```python
from build123d import *

# Parameters (mm, degrees)
CUT_EXTRUDE1_DEPTH      = 124.693168769
CUT_EXTRUDE1_DEPTH_BACK = 124.693168769
CUT_EXTRUDE2_DEPTH      = 124.693168769


with BuildPart() as part:
    # Sketch1 → Revolve2 (revolve)
    with BuildSketch(Plane(origin=(0, 0, 0), x_dir=(0, 0, -1), z_dir=(1, 0, 0))):
        Polygon((-50, 64), (-50, 80), (0, 80), (0, 0), (-30, 0), (-30, 64), align=None)
    revolve(axis=Axis((0, 0, -85.976986238), (0, 0, 1)))

    # Sketch2 → Cut-Extrude1 (cut, two sides: drawn at the far end of the back side and taken through both)
    with BuildSketch(Plane(origin=(0, 0, 0), x_dir=(0, 0, -1), z_dir=(1, 0, 0)).offset(-CUT_EXTRUDE1_DEPTH_BACK)):
        Polygon((-50, 80), (-38.811710089, 80), (-50, -80), align=None)
    extrude(amount=CUT_EXTRUDE1_DEPTH + CUT_EXTRUDE1_DEPTH_BACK, mode=Mode.SUBTRACT)

    # Sketch3 → Cut-Extrude2 (cut, through all)
    with BuildSketch(Plane.XY):
        with BuildLine():
            Line((30, 15), (30, -100))
            ThreePointArc((30, -100), (0, -130), (-30, -100))
            Line((-30, -100), (-30, 15))
            ThreePointArc((-30, 15), (0, 45), (30, 15))
        make_face()
    extrude(amount=CUT_EXTRUDE2_DEPTH, mode=Mode.SUBTRACT)


solid = part.part
```
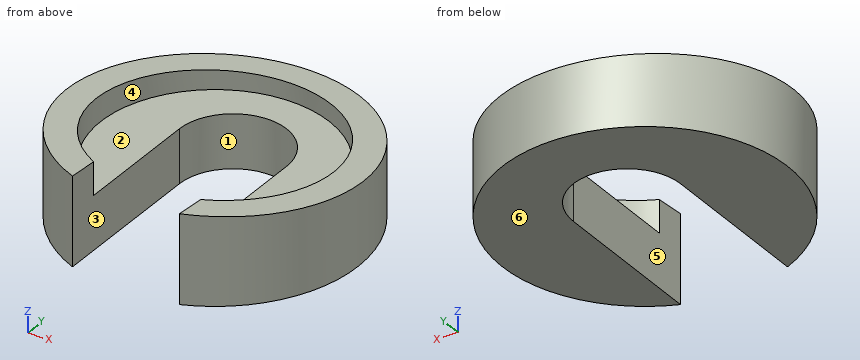
Input: part model. Units: mm. Frame: model coordinates. Face numbers are marked on the shaded views. A direction names the side the tool comes from. Give positions to 0.01 mm unless a question says otherwise; leave off trailing zeros. Order: outer loops, then holes, each group sorted by start corner. A loop starts at its lowest first (then second) coordinate and runs counter-clockwise, first axis right, second up.
1. Cut plane D-D (y = 35). Return loops of the section in (x, z).
Computed:
outline: (-71.94, 0) - (-22.36, 0) - (-22.36, 30) - (-53.58, 30) - (-53.58, 41.96) - (-71.94, 41.96) - close; (22.36, 0) - (71.94, 0) - (71.94, 41.96) - (53.58, 41.96) - (53.58, 30) - (22.36, 30) - close
2. Draft query along Y for the marked faces 1, 2 and 3. Return one class per face: released by +Y, released by -Y, zero draft, split by the parting line, or undercut.
Computed:
face 1: released by -Y
face 2: undercut
face 3: zero draft
3. Cut plane C-C (x = 19.5). Return loops of the section in (y, z).
Computed:
outline: (37.8, 0) - (77.59, 0) - (77.59, 38.98) - (60.96, 40.14) - (60.96, 30) - (37.8, 30) - close
4. Cut plane B-B (z = 25.5). Return loops of the section in (x, y), and give its area (3 significant figures).
Computed:
outline: (-30, -74.16) - (-30, 15) arc R30 cw to (30, 15) - (30, -74.16) arc R80 ccw (long way) to start
area: 13,100 mm2
5. Line query: probe 1 along X at (y, z) = (0, 39); probe 2 along X at (y, z) = (1, 6.5); probe 3 along Y at (x, z) = (0, 35). Output: solid intervals per line, ascending.
Computed:
probe 1: x = -80 to -64, 64 to 80
probe 2: x = -79.99 to -30, 30 to 79.99
probe 3: y = 64 to 80
6. Set-up query: the marked faces 4, 5 and 6. Return all of +Z, -Z, +X, -X, +Y, -Y with unobstructed straight access to the full face (end or side cutting, diameter ignored); none if empty.
Computed:
face 4: +Z
face 5: +Z, -Z, -Y
face 6: -Z, +X, -X, +Y, -Y
7. Cut plane A-A (y = -63). Return loops of the section in (x, z), and give its area (3 significant figures).
Computed:
outline: (-49.31, 0) - (-30, 0) - (-30, 48.81) - (-49.31, 48.81) - close; (30, 0) - (49.31, 0) - (49.31, 48.81) - (30, 48.81) - close
area: 1,880 mm2
8. Pin query (flat end, axial travel): pin 1 Ø1.5 at (y, z) = (48, 18) entering from +X; pin 2 Ø4 at (x, z) = (22, 43.5) entering from +Y; pin 3 Ø8 at (x, y) = (-54.5, -12.5) entering from +Z; pin 4 Ø3 at (x, y) = (-53, 5) entering from -Z. Return the tip coordinate at first contact, or that it passes through.
Computed:
pin 1: stops at x = 64.56
pin 2: passes through
pin 3: stops at z = 30
pin 4: stops at z = 0
